Design review of the part built by this model. Coordinates are the model's own, in mm. A direction names the side the tool comes from. Give positions to 0.01 mm unless a question says otherwise; leave off trailing zeros. Write each loop counter-clockwise with the first axis right and the second up, starting at its lowest first coordinate (ties: lowest second). Pieces come first, ordered by that corner, then holes. Notation, with made-up numbers: M -29,34.5 L -7,34.5 A32 ccw -7,70.5 Z; hole C 86,-3.75 d9. An arc over 180 degrees is marked long. Answer in a Markdown table with one row per item.
```python
from build123d import *

# Parameters (mm, degrees)
SKETCH1_W                                          = 70
SKETCH1_H                                          = 200
BOSS_EXTRUDE1_DEPTH                                = 14
HOLE_SIZE_BASED_ON_SOCKET_HEAD_CAP_SCR_D           = 9
HOLE_SIZE_BASED_ON_SOCKET_HEAD_CAP_SCR_CBORE_D     = 15
HOLE_SIZE_BASED_ON_SOCKET_HEAD_CAP_SCR_CBORE_DEPTH = 9
HOLE_SIZE_BASED_ON_SOCKET_HEAD_CAP_2_D             = 9
HOLE_SIZE_BASED_ON_SOCKET_HEAD_CAP_2_CBORE_D       = 15
HOLE_SIZE_BASED_ON_SOCKET_HEAD_CAP_2_CBORE_DEPTH   = 9


with BuildPart() as part:
    # Sketch1 → Boss-Extrude1 (new body)
    with BuildSketch(Plane(origin=(0, 0, 0), x_dir=(1, 0, 0), z_dir=(0, 1, 0))):
        with Locations((35, 100)):
            Rectangle(SKETCH1_W, SKETCH1_H)
    extrude(amount=BOSS_EXTRUDE1_DEPTH)

    # Hole size _based on_ socket head cap scr (through all)
    with Locations(Plane(origin=(0, 14, 0), x_dir=(1, 0, 0), z_dir=(0, 1, 0))):
        with Locations((10, 155), (60, 155), (60, 45), (10, 45)):
            CounterBoreHole(HOLE_SIZE_BASED_ON_SOCKET_HEAD_CAP_SCR_D / 2, HOLE_SIZE_BASED_ON_SOCKET_HEAD_CAP_SCR_CBORE_D / 2, HOLE_SIZE_BASED_ON_SOCKET_HEAD_CAP_SCR_CBORE_DEPTH)

    # Hole size _based on_ socket head cap 2 (through all)
    with Locations(Plane(origin=(0, 0, 0), x_dir=(-1, 0, 0), z_dir=(0, -1, 0))):
        with Locations((-60, 188), (-10, 188), (-10, 12), (-60, 12)):
            CounterBoreHole(HOLE_SIZE_BASED_ON_SOCKET_HEAD_CAP_2_D / 2, HOLE_SIZE_BASED_ON_SOCKET_HEAD_CAP_2_CBORE_D / 2, HOLE_SIZE_BASED_ON_SOCKET_HEAD_CAP_2_CBORE_DEPTH)


solid = part.part
```
1) To check wall thickness, follow probe 1 along Z at (x, y) = (60, 2.9); probe 2 along X at (y, z) = (10, -155); probe 3 along X at (y, z) = (1.7, -155). State the ranges of each line that lie inside material, in increasing order. Write a range as [from, to].
Geometry says:
| item | result |
|---|---|
| probe 1 | [-200, -195.5], [-180.5, -159.5], [-150.5, -49.5], [-40.5, -19.5], [-4.5, 0] |
| probe 2 | [0, 2.5], [17.5, 52.5], [67.5, 70] |
| probe 3 | [0, 5.5], [14.5, 55.5], [64.5, 70] |
2) For faces 1 (the face through (59.024, 9.563, -162.436)), 2 (the face through (35, 14, -101)), 3 (the face through (65.952, 4.437, -7.436)), list the 3-axis set-ups (+Z, -Z, +X, -X, +Y, -Y) from which the entire face can be reached by the end or side of a thin tool; tool diameter is ignored.
Geometry says:
| item | result |
|---|---|
| face 1 | +Y |
| face 2 | +Z, -Z, +X, -X, +Y |
| face 3 | -Y |
3) The part is to be moulded in two halves that separate along Z. For faces 4 (the face through (35, 7, 0)), 5 (the face through (11.63, 4.44, -4.68)), 6 (the face through (70, 7, -99)), 7 (the face through (35, 7, -200)), say which applies: released by +Z, released by -Z, zero draft, split by the parting line, or undercut.
Geometry says:
| item | result |
|---|---|
| face 4 | released by +Z |
| face 5 | undercut |
| face 6 | zero draft |
| face 7 | released by -Z |
4) Add section B-B (z = -45). Write out the cut boundary in (x, y), and give its area (3 significant figures).
Geometry says:
| item | result |
|---|---|
| outline | M 0,0 L 5.5,0 L 5.5,5 L 2.5,5 L 2.5,14 L 0,14 Z; M 14.5,0 L 55.5,0 L 55.5,5 L 52.5,5 L 52.5,14 L 17.5,14 L 17.5,5 L 14.5,5 Z; M 64.5,0 L 70,0 L 70,14 L 67.5,14 L 67.5,5 L 64.5,5 Z |
| area | 620 mm^2 |
5) Insertion check: P1, Ø2, axis at y = 2, z = -168, coming from the -X side; P2, Ø13.5, axis at x = 60, z = -12, coming from the -Y side; P3, Ø7.5, axis at x = 61.5, z = -47.5, coming from the +Y side. Each pin has a flat end and moves straight along its axis. Give the tip position at first contact, or say it passes through.
Geometry says:
| item | result |
|---|---|
| P1 | x = 0 |
| P2 | y = 9 |
| P3 | y = 5 |
6) Add section A-A (y = 3). Count the separate pieces of the cut face and the enclosed holes in it, and give its area (3 significant figures).
Geometry says:
| item | result |
|---|---|
| separate pieces | 1 |
| enclosed holes | 8 |
| area | 13,000 mm^2 |
